```python
from build123d import *

# Parameters (mm, degrees)
HOT_ROLLED_UNEQUAL_ANGLE_GB_T706_2008_10_DEPTH = 100
SKETCH3_OUTSIDE_W                              = 132.964
SKETCH3_OUTSIDE_H                              = 132.964
CUT_EXTRUDE1_DEPTH                             = 10
CUT_EXTRUDE2_DEPTH                             = 15


with BuildPart() as part:
    # Sketch1 → Hot-rolled unequal angle gb∕t706-2008 100 X 63 X 6(1) (new body)
    with BuildSketch(Plane(origin=(0, 0, 0), x_dir=(0, 0, -1), z_dir=(1, 0, 0))):
        with BuildLine():
            Line((0, 0), (0, 100))
            Line((0, 100), (2.666666667, 100))
            ThreePointArc((2.666666667, 100), (5.023689271, 99.023689271), (6, 96.666666667))
            Line((6, 96.666666667), (6, 16))
            ThreePointArc((6, 16), (8.928932188, 8.928932188), (16, 6))
            Line((16, 6), (59.666666667, 6))
            ThreePointArc((59.666666667, 6), (62.023689271, 5.023689271), (63, 2.666666667))
            Line((63, 2.666666667), (63, 0))
            Line((63, 0), (0, 0))
        make_face()
    extrude(amount=HOT_ROLLED_UNEQUAL_ANGLE_GB_T706_2008_10_DEPTH)

    # Sketch3 outside → Cut-Extrude1 (cut)
    # profile 1 of 2: a face of its own
    with BuildSketch(Plane.XY):
        with Locations((50, 50)):
            Rectangle(SKETCH3_OUTSIDE_W, SKETCH3_OUTSIDE_H)
        with BuildLine():
            Line((0, 30), (17.101007166, 76.984631039))
            ThreePointArc((17.101007166, 76.984631039), (50, 100.040750994), (82.898992834, 76.984631039))
            Line((82.898992834, 76.984631039), (100, 30))
            Line((100, 30), (100, 0))
            Line((100, 0), (0, 0))
            Line((0, 0), (0, 30))
        make_face(mode=Mode.SUBTRACT)
    # profile 2 of 2: a face of its own
    with BuildSketch(Plane.XY):
        with BuildLine():
            Line((59, 80), (59, 60))
            ThreePointArc((59, 60), (50, 51), (41, 60))
            Line((41, 60), (41, 80))
            ThreePointArc((41, 80), (50, 89), (59, 80))
        make_face()
    extrude(amount=-CUT_EXTRUDE1_DEPTH, mode=Mode.SUBTRACT)

    # Sketch4 → Cut-Extrude2 (cut)
    with BuildSketch(Plane.XZ):
        with BuildLine():
            Line((20.5, -20), (20.5, -50))
            ThreePointArc((20.5, -50), (15, -55.5), (9.5, -50))
            Line((9.5, -50), (9.5, -20))
            ThreePointArc((9.5, -20), (15, -14.5), (20.5, -20))
        make_face()
        with BuildLine():
            Line((79.5, -20), (79.5, -50))
            ThreePointArc((79.5, -50), (85, -55.5), (90.5, -50))
            Line((90.5, -50), (90.5, -20))
            ThreePointArc((90.5, -20), (85, -14.5), (79.5, -20))
        make_face()
    extrude(amount=-CUT_EXTRUDE2_DEPTH, mode=Mode.SUBTRACT)


solid = part.part
```
Design review of the part built by this model. Coordinates are the model's own, in mm. A direction names the side the tool comes from. Give positions to 0.01 mm unless a question says otherwise; leave off trailing zeros. Loops run counter-clockwise (first coordinate to the right, second up) from the corner with the lowest first, then second, coordinate; pieces in that order, holes last. Notation, with made-up numbers: (24.25, -0.5) -> (67.25, -0.5) arc R22 ccw to (67.25, 31.5) -> close; hole circle Ø5 at (-4.5, -24). An arc over 180 degrees is marked (long way). Write each question's results on one line, items separated by ' | '.
Q1. Wall thickness on L1, parallel to Y at x = 56, z = -21; L2, parallel to Z at x = 8, y = 31; L3, parallel to Y at x = 90.5, z = -8: over which ranges is each line inside the solid? List them lowest first.
Reply:
L1: y = 0 to 6 | L2: z = -6 to 0 | L3: y = 0 to 10
Q2. Take a section at A-A, the plane z = -32. Write out the cut boundary in (x, y).
Reply:
outline: (0, 0) -> (9.5, 0) -> (9.5, 6) -> (0, 6) -> close; (20.5, 0) -> (79.5, 0) -> (79.5, 6) -> (20.5, 6) -> close; (90.5, 0) -> (100, 0) -> (100, 6) -> (90.5, 6) -> close
Q3. Take a section at B-B, the plane x = 50. Write out the cut boundary in (y, z), plus the area to 3 significant figures.
Reply:
outline: (0, -63) -> (2.67, -63) arc R3.33 ccw to (6, -59.67) -> (6, -16) arc R10 cw to (16, -6) -> (51, -6) -> (51, 0) -> (0, 0) -> close; (89, -6) -> (96.67, -6) arc R3.33 ccw to (100, -2.67) -> (100, 0) -> (89, 0) -> close | area: 731 mm²
Q4. The part is to be moulded in two halves that separate along Z. For faces 5 (the face through (49.79, 98.608, -5.376)), 6 (the face through (49, 38, 0)), 7 (the face through (8.43, 53.16, -2.96)), 8 (the face through (90.5, 3, -35)), say which applies: +Z half, -Z half, draft (parallel to the pull), parting line (faces both ways), or undercut.
Reply:
face 5: -Z half | face 6: +Z half | face 7: draft | face 8: undercut
Q5. Take a section at C-C, the plane y = 71. Write out the cut boundary in (x, z).
Reply:
outline: (14.92, -6) -> (41, -6) -> (41, 0) -> (14.92, 0) -> close; (59, -6) -> (85.08, -6) -> (85.08, 0) -> (59, 0) -> close
Q6. Machinability: for faces 1 (the face through (79.5, 3, -35)), 2 (the face through (41, 70, -3)), 3 (the face through (70.54, 93.38, -2.96)), 4 (the face through (49, 6, -38)), which of the approach directions +Z, -Z, +X, -X, +Y, -Y give a long, thin tool a straight path to every point of the face, cutting with its end or side? Answer none if there is none.
Reply:
face 1: +Y, -Y | face 2: +Z, -Z | face 3: +Z, -Z, +X, +Y | face 4: -Z, +X, -X, +Y
Q7. Take a section at D-D, the plane x = 23. Write out the cut boundary in (y, z), plus the area to 3 significant figures.
Reply:
outline: (0, -63) -> (2.67, -63) arc R3.33 ccw to (6, -59.67) -> (6, -16) arc R10 cw to (16, -6) -> (87.31, -6) -> (87.31, 0) -> (0, 0) -> close | area: 885 mm²
Q8. For pin 1 Ø6.5 at (y, z) = (69, -4) entering from -X; pin 2 Ø10 at (y, z) = (65, -7.5) entering from +X; pin 3 Ø1.5 at (x, y) = (33.5, 38) entering from -Z, all flat-tipped, find the tip position at first contact; note any pin that passes through.
Reply:
pin 1: stops at x = 13.01 | pin 2: stops at x = 89 | pin 3: stops at z = -6
